Check sheet for the modelled part. Datum: model origin and axes. Units: mm. Face numbers are marked on the shaded views. A direction names the side the tool comes from. Coordinates: 2 decimals unless noted, no trailing zeros. Write each loop counter-clockwise with the first axis right and the second up, starting at its lowest first coordinate (ties: lowest second). Pieces come first, ordered by that corner, then holes. Notation, with made-up numbers: (27, 71.25) - (81, 71.25) arc R27 cw to (81, 104.25) - close; hole circle Ø7 at (82.5, -6). An arc over 180 degrees is marked (long way). Use one line per item in the form item = value. Start each with the question number.
1. Tool access check on the marked faces 4, 5, 6, 7 and 8. Record the directions out of +Z, -Z, +X, -X, +Y, -Y that give a thin tool (end or side, any length) a straight path to the whole face; none if there is none.
2. Cross-section at C-C on x = 4. Record the boundary of the cut face in (y, z).
3. Cross-section at D-D on z = 17.75. Record the boundary of the cut face in (x, y), then the cut area to 4 significant figures.
4. Scan lines: line 1 along Z through (x, y) = (4, 1); line 2 along X through (y, z) = (-12.5, 10); line 3 along Y through (x, z) = (38, 8.5). Record each from-to range of solid material in increasing order.
5. Cross-section at B-B on z = 10. Record the boundary of the cut face in (x, y).
6. Draft check along X on the marked faces 1, 2 and 3. Enter one of: +X half, -X half, draft (parallel to the pull), parting line (faces both ways), or undercut.
7. Go/stop test with flat-tipped pins: pin 1 Ø10 at (x, z) = (42, 8.5) entering from +Y; pin 2 Ø2 at (y, z) = (-19, 6.5) entering from -X; pin 3 Ø6 at (y, z) = (-16, 16.5) entering from -X. Record where each tip stops, or that it passes through.
8. Cross-section at A-A on x = 31.5. Record the boundary of the cut face in (y, z).
```python
from build123d import *

# Parameters (mm, degrees)
BASE_BLOCK_DEPTH         = 20
END_LUGS_DEPTH           = 20
GUIDE_V_SLOT_DEPTH       = 63
LOCATING_PIN_SKETCH_14_R = 7
LOCATING_PIN_14_DEPTH    = 15
HOLE_SKETCH_8_R          = 4
HOLE_8_DEPTH             = 32


with BuildPart() as part:
    # Base Profile Sketch → Base Block (new body)
    with BuildSketch(Plane.XY):
        Polygon((0, 0), (63, 0), (63, -5), (48.5, -12), (31.5, -12), (14.5, -12), (0, -5), align=None)
    extrude(amount=BASE_BLOCK_DEPTH)

    # End Lugs Sketch → End Lugs (add)
    with BuildSketch(Plane.XY.offset(20)):
        Polygon((0, 0), (0, 5), (7.5, 5), (14.5, 0), align=None)
        Polygon((63, 0), (63, 5), (55.5, 5), (48.5, 0), align=None)
    extrude(amount=-END_LUGS_DEPTH)

    # Guide V-Slot Sketch → Guide V-Slot (cut)
    with BuildSketch(Plane.ZY):
        Polygon((10, 5), (6.5, 5), (6.5, 0), (13.5, 0), (13.5, 5), align=None)
    extrude(amount=-GUIDE_V_SLOT_DEPTH, mode=Mode.SUBTRACT)

    # Locating Pin Sketch Ø14 → Locating Pin Ø14 (add)
    with BuildSketch(Plane.XZ.offset(12)):
        with Locations(Location((31.5, 10, 0), (0, 0, 270))):
            Circle(LOCATING_PIN_SKETCH_14_R)
    extrude(amount=LOCATING_PIN_14_DEPTH)

    # Hole Sketch Ø8 → Hole Ø8 (cut)
    with BuildSketch(Plane(origin=(0, 0, 0), x_dir=(1, 0, 0), z_dir=(0, 1, 0))):
        with Locations(Location((31.5, -10, 0), (0, 0, 270))):
            Circle(HOLE_SKETCH_8_R)
    extrude(amount=-HOLE_8_DEPTH, mode=Mode.SUBTRACT)


solid = part.part
```
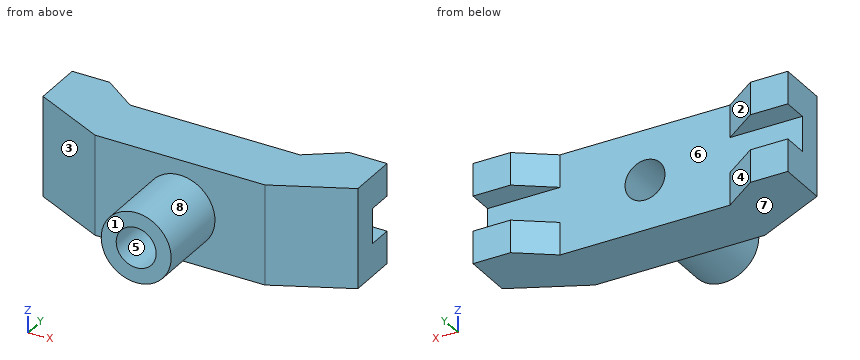
Final values:
q1.face_4 = +Z, -Z, +Y
q1.face_5 = +Y, -Y
q1.face_6 = +Y
q1.face_7 = -Z, +X, -X, +Y, -Y
q1.face_8 = -Y
q2.outline = (-6.93, 0) - (5, 0) - (5, 6.5) - (0, 6.5) - (0, 13.5) - (5, 13.5) - (5, 20) - (-6.93, 20) - close
q3.outline = (0, -5) - (14.5, -12) - (48.5, -12) - (63, -5) - (63, 5) - (55.5, 5) - (48.5, 0) - (14.5, 0) - (7.5, 5) - (0, 5) - close
q3.area = 764.5 mm²
q4.line_1 = 0 to 6.5, 13.5 to 20
q4.line_2 = 24.5 to 27.5, 35.5 to 38.5
q4.line_3 = -27 to 0
q5.outline = (0, -5) - (14.5, -12) - (24.5, -12) - (24.5, -27) - (27.5, -27) - (27.5, 0) - (0, 0) - close; (35.5, -27) - (38.5, -27) - (38.5, -12) - (48.5, -12) - (63, -5) - (63, 0) - (35.5, 0) - close
q6.face_1 = draft
q6.face_2 = undercut
q6.face_3 = -X half
q7.pin_1 = 0
q7.pin_2 = 24.96
q7.pin_3 = 25.44
q8.outline = (-27, 3) - (-12, 3) - (-12, 0) - (0, 0) - (0, 6) - (-27, 6) - close; (-27, 14) - (0, 14) - (0, 20) - (-12, 20) - (-12, 17) - (-27, 17) - close
